Geometry check sheet. Reference: the model listing, model coordinates, mm. A direction names the side the tool comes from. Coordinates: 2 decimals unless noted, no trailing zeros. Order: outer loops, then holes, each group sorted by start corner. A loop starts at its lowest first (then second) coordinate and runs counter-clockwise, first axis right, second up. Notation, with made-up numbers: (-26, -26.75) - (11, -26.75) arc R27 ccw to (11, -2.75) - close; hole circle Ø8 at (13, -2). An arc over 180 degrees is marked (long way). Return JSON: item names as keys, results as strings. Group by question number.
Item 1: Section check A-A on y = 3.4. Enter the section's corners in (x, z), then the cut area to 3 significant figures.
Item 2: Section check C-C on x = 1. Enter the section's corners in (y, z).
Item 3: Scan lines: probe 1 along Y at (x, z) = (-2.75, -2.5); probe 2 along X at (y, z) = (3.9, -5.5); probe 3 along X at (y, z) = (5.55, -6.5). Record each from-to range of solid material in increasing order.
Item 4: Tool access check on faces 1 (the flat face through (2, 4.4, 0)), 2 (the flat face through (1.75, 5, 0)), 3 (the flat face through (4.5, 3, 0)). Record the directions out of +Z, -Z, +X, -X, +Y, -Y that give a thin tool (end or side, any length) a straight path to the whole face; none if there is none.
Item 5: Draft check along Y on faces 4 (the flat face through (0, 0, 0)), 5 (the flat face through (0, 1, 25)), 6 (the flat face through (3, 6, 0)), 7 (the flat face through (-2, 4.4, 0)). Enter one of: pulls with the +Y half, pulls with the -Y half, needs draft (parallel to the pull), parting line crosses it, or undercut.
Item 6: Section check B-B on z = 22.5. Enter the section's corners in (x, y).
Item 7: Gauge pin test, flat end, axial feed: pin 1 (0.6 mm diameter, centred on x = -2.5, z = -9.5, fed in from -Y). Record the tip position at first contact, or that the pin passes through.
from build123d import *

# Parameters (mm, degrees)
EXTRUDE_1_DEPTH = 25


with BuildPart() as part:
    # 草图1 → 凸台-拉伸1 (new, symmetric)
    with BuildSketch(Plane.XY):
        Polygon((0, 0), (-4.5, 0), (-4.5, 6), (-1.75, 6), (-1.75, 4.4), (-2.9, 4.4), (-2.9, 1.6), (2.9, 1.6), (2.9, 4.4), (1.75, 4.4), (1.75, 6), (4.5, 6), (4.5, 0), align=None)
    extrude(amount=EXTRUDE_1_DEPTH, both=True)


solid = part.part
Computed:
{
 "1": {"outline": "(-4.5, -25) - (-2.9, -25) - (-2.9, 25) - (-4.5, 25) - close; (2.9, -25) - (4.5, -25) - (4.5, 25) - (2.9, 25) - close", "area": "160 mm²"},
 "2": {"outline": "(0, -25) - (1.6, -25) - (1.6, 25) - (0, 25) - close"},
 "3": {"probe 1": "y = 0 to 1.6, 4.4 to 6", "probe 2": "x = -4.5 to -2.9, 2.9 to 4.5", "probe 3": "x = -4.5 to -1.75, 1.75 to 4.5"},
 "4": {"face 1": "+Z, -Z", "face 2": "+Z, -Z, +Y", "face 3": "+Z, -Z, +X, +Y, -Y"},
 "5": {"face 4": "pulls with the -Y half", "face 5": "needs draft", "face 6": "pulls with the +Y half", "face 7": "undercut"},
 "6": {"outline": "(-4.5, 0) - (4.5, 0) - (4.5, 6) - (1.75, 6) - (1.75, 4.4) - (2.9, 4.4) - (2.9, 1.6) - (-2.9, 1.6) - (-2.9, 4.4) - (-1.75, 4.4) - (-1.75, 6) - (-4.5, 6) - close"},
 "7": {"pin 1": "stops at y = 0"}
}
